CAD build for the part. Positions are in the model's coordinates, mm. A direction names the side the tool comes from. Give positions to 0.01 mm unless a question says otherwise; leave off trailing zeros. Write each loop counter-clockwise with the first axis right and the second up, starting at its lowest first coordinate (ties: lowest second). Pieces come first, ordered by that corner, then holes. Notation, with made-up numbers: (16.25, 70) - (44.25, 70) arc R19 ccw to (44.25, 78) - close; hole circle Ø5 at (-9, 78). An arc over 180 degrees is marked (long way). Answer as a JSON object with one key per item and string values.
from build123d import *

# Parameters (mm, degrees)
SKETCH_1_W               = 60
SKETCH_1_H               = 40
EXTRUDE_1_DEPTH          = 21
SKETCH_2_W               = 40
SKETCH_2_H               = 46.112845628
CUT_EXTRUDE_1_DEPTH      = 12
SKETCH_3_W               = 80.513519028
SKETCH_3_H               = 24
CUT_EXTRUDE_2_DEPTH      = 12
SKETCH_4_W               = 4.5
SKETCH_4_H               = 30.3
CUT_EXTRUDE_3_DEPTH      = 67.640828326
SKETCH_5_R               = 2.25
CUT_EXTRUDE_4_DEPTH      = 12
MIRROR_2_COPY_1_SKETCH_R = 2.25
MIRROR_2_COPY_1_DEPTH    = 12
CUT_EXTRUDE_5_DEPTH      = 4
MIRROR_4_COPY_1_DEPTH    = 4
SKETCH_7_R               = 0.5
CUT_EXTRUDE_6_DEPTH      = 67.640828326
CHAMFER_1_SIZE           = 0.5


with BuildPart() as part:
    # 草图1 → 凸台-拉伸1 (new body)
    with BuildSketch(Plane.XY):
        Rectangle(SKETCH_1_W, SKETCH_1_H)
    extrude(amount=EXTRUDE_1_DEPTH)

    # 草图2 → 切除-拉伸1 (cut)
    with BuildSketch(Plane.XY.offset(21)):
        Rectangle(SKETCH_2_W, SKETCH_2_H)
    extrude(amount=-CUT_EXTRUDE_1_DEPTH, mode=Mode.SUBTRACT)

    # 草图3 → 切除-拉伸2 (cut)
    with BuildSketch(Plane.XY.offset(21)):
        Rectangle(SKETCH_3_W, SKETCH_3_H)
    extrude(amount=-CUT_EXTRUDE_2_DEPTH, mode=Mode.SUBTRACT)

    # 草图4 → 切除-拉伸3 (cut, through all)
    with BuildSketch(Plane.ZY.offset(30)):
        with Locations((14.25, 0)):
            Rectangle(SKETCH_4_W, SKETCH_4_H)
    extrude(amount=-CUT_EXTRUDE_3_DEPTH, mode=Mode.SUBTRACT)

    # 草图5 → 切除-拉伸4 (cut)
    with BuildSketch(Plane.XY.offset(9)):
        with Locations((-13, 13)):
            Circle(SKETCH_5_R)
    cut_extrude_4 = extrude(amount=-CUT_EXTRUDE_4_DEPTH, mode=Mode.SUBTRACT)

    # 镜向1: 切除-拉伸4 across plane
    add(cut_extrude_4.mirror(Plane.ZX), mode=Mode.SUBTRACT)

    # 镜向2: 切除-拉伸4 across plane
    add(cut_extrude_4.mirror(Plane(origin=(0, 0, 0), x_dir=(0, 0, 1), z_dir=(1, 0, 0))), mode=Mode.SUBTRACT)

    # 镜向2 copy 1 sketch → 镜向2 copy 1 (cut)
    with BuildSketch(Plane(origin=(0, 0, 9), x_dir=(-1, 0, 0), z_dir=(0, 0, 1))):
        with Locations((-13, 13)):
            Circle(MIRROR_2_COPY_1_SKETCH_R)
    extrude(amount=-MIRROR_2_COPY_1_DEPTH, mode=Mode.SUBTRACT)

    # 草图6 → 切除-拉伸5 (cut)
    with BuildSketch(Plane.XY.offset(9)):
        Polygon((-8.958548116, 13), (-10.979274058, 16.5), (-15.020725942, 16.5), (-17.041451884, 13), (-15.020725942, 9.5), (-10.979274058, 9.5), align=None)
    cut_extrude_5 = extrude(amount=-CUT_EXTRUDE_5_DEPTH, mode=Mode.SUBTRACT)

    # 镜向3: 切除-拉伸5 across plane
    add(cut_extrude_5.mirror(Plane(origin=(0, 0, 0), x_dir=(0, 0, 1), z_dir=(1, 0, 0))), mode=Mode.SUBTRACT)

    # 镜向4: 切除-拉伸5 across plane
    add(cut_extrude_5.mirror(Plane.ZX), mode=Mode.SUBTRACT)

    # 镜向4 copy 1 sketch → 镜向4 copy 1 (cut)
    with BuildSketch(Plane(origin=(0, 0, 9), x_dir=(-1, 0, 0), z_dir=(0, 0, 1))):
        Polygon((-8.958548116, 13), (-10.979274058, 16.5), (-15.020725942, 16.5), (-17.041451884, 13), (-15.020725942, 9.5), (-10.979274058, 9.5), align=None)
    extrude(amount=-MIRROR_4_COPY_1_DEPTH, mode=Mode.SUBTRACT)

    # 草图7 → 切除-拉伸6 (cut, through all)
    with BuildSketch(Plane.ZY.offset(30)):
        with Locations((12.2, 15.05)):
            Circle(SKETCH_7_R)
        with Locations((16.5, 15.15)):
            Circle(SKETCH_7_R)
    cut_extrude_6 = extrude(amount=-CUT_EXTRUDE_6_DEPTH, mode=Mode.SUBTRACT)

    # 镜向5: 切除-拉伸6 across plane
    add(cut_extrude_6.mirror(Plane.ZX), mode=Mode.SUBTRACT)

    # 倒角1
    chamfer_1_edges = [part.edges().sort_by_distance(p)[0] for p in [
        (-25, 20, 21),
        (25, -20, 21),
        (-25, -20, 21),
        (25, 20, 21),
    ]]
    chamfer(chamfer_1_edges, length=CHAMFER_1_SIZE)


solid = part.part
(1) Pull direction Z, two halves, no side cores. Call faces 1 (the face through (-25, 13, 16.5)), 2 (the face through (-11, -15, 5)), 3 (the face through (-10, 11.2, 7)): pulls with the +Z half, pulls with the -Z half, needs draft (parallel to the pull), parting line crosses it, or undercut.
Answer key:
{"face 1": "undercut", "face 2": "pulls with the +Z half", "face 3": "needs draft"}
(2) Saw through at A-A, the plane z = 18. Give the cut face in (x, y), and give its area (3 significant figures).
Answer key:
{"outline": "(-30, -20) - (-20, -20) - (-20, -12) - (-30, -12) - close; (-30, 12) - (-20, 12) - (-20, 20) - (-30, 20) - close; (20, -20) - (30, -20) - (30, -12) - (20, -12) - close; (20, 12) - (30, 12) - (30, 20) - (20, 20) - close", "area": "320 mm²"}
(3) Saw through at B-B, the plane z = 6.75. Give the cut face in (x, y).
Answer key:
{"outline": "(-30, -20) - (30, -20) - (30, 20) - (-30, 20) - close; hole (-17.04, -13) - (-15.02, -16.5) - (-10.98, -16.5) - (-8.96, -13) - (-10.98, -9.5) - (-15.02, -9.5) - close; hole (-17.04, 13) - (-15.02, 9.5) - (-10.98, 9.5) - (-8.96, 13) - (-10.98, 16.5) - (-15.02, 16.5) - close; hole (8.96, -13) - (10.98, -16.5) - (15.02, -16.5) - (17.04, -13) - (15.02, -9.5) - (10.98, -9.5) - close; hole (8.96, 13) - (10.98, 9.5) - (15.02, 9.5) - (17.04, 13) - (15.02, 16.5) - (10.98, 16.5) - close"}
(4) Flat gauge pins, fed straight in: P1, Ø5, axis at x = -13, y = -13, coming from the +Z side; P2, Ø20, axis at x = 3, y = -5.5, coming from the +Z side. Where does each tip first touch, or does it go through?
Answer key:
{"P1": "stops at z = 5", "P2": "stops at z = 9"}
(5) 3-axis set-ups, long thin cutter, end or side, ignore diameter. For faces 4 (the face through (16.045, -11.274, 7.028)), 5 (the face through (-25, 15.15, 14)), 6 (the face through (-25, 12, 19)): which of +Z, -Z, +X, -X, +Y, -Y reach the whole face in a straight line?
Answer key:
{"face 4": "+Z", "face 5": "+X, -X", "face 6": "+Z, +X, -X"}
(6) Saw through at C-C, the plane x = -13. Give the cut face in (y, z), and give its area (3 significant figures).
Answer key:
{"outline": "(-20, 0) - (-15.25, 0) - (-15.25, 5) - (-16.5, 5) - (-16.5, 9) - (-20, 9) - close; (-10.75, 0) - (10.75, 0) - (10.75, 5) - (9.5, 5) - (9.5, 9) - (-9.5, 9) - (-9.5, 5) - (-10.75, 5) - close; (15.25, 0) - (20, 0) - (20, 9) - (16.5, 9) - (16.5, 5) - (15.25, 5) - close", "area": "259 mm²"}
(7) Saw through at D-D, the plane z = 2.5. Give the cut face in (x, y).
Answer key:
{"outline": "(-30, -20) - (30, -20) - (30, 20) - (-30, 20) - close; hole circle Ø4.5 at (-13, -13); hole circle Ø4.5 at (-13, 13); hole circle Ø4.5 at (13, -13); hole circle Ø4.5 at (13, 13)"}
(8) Probe L1, parallel to Y at x = 13, z = 3.7; L2, parallel to X at y = 18.5, z = 9.75; L3, parallel to X at y = 11, z = 3.5. List the from-to ranges inside material, lowest first. Write a range as [from, to].
Answer key:
{"L1": "y = [-20, -15.25], [-10.75, 10.75], [15.25, 20]", "L2": "x = [-30, -20], [20, 30]", "L3": "x = [-30, -14.03], [-11.97, 11.97], [14.03, 30]"}
